from build123d import *

# Parameters (mm, degrees)
BASE_PLATE_DEPTH         = 12
LUG_DEPTH                = 35
BOSS_SKETCH_R            = 25
CYLINDRICAL_BOSS_DEPTH   = 45
LUG_FILLET_R6_R          = 6
MIRRORED_LUG_FILLET_R6_R = 6
BOSS_BORE_SKETCH_R       = 16
BOSS_BORE_DEPTH          = 131
SIDE_EAR_SKETCH_R        = 10.000000003
SIDE_EAR_DEPTH           = 10
RELIEF_CUT_SKETCH_R      = 5
RELIEF_CUT_DEPTH         = 10


with BuildPart() as part:
    # Base Plate Sketch → Base Plate (new body)
    with BuildSketch(Plane(origin=(0, 0, 0), x_dir=(1, 0, 0), z_dir=(0, 1, 0))):
        with BuildLine():
            Line((0, 0), (52.086042587, 0))
            Line((52.086042587, 0), (52.086042587, 34.268491931))
            ThreePointArc((52.086042587, 34.268491931), (55.457925039, 42.608491187), (63.678640518, 46.261574252))
            ThreePointArc((63.678640518, 46.261574252), (70.963844757, 49.044672415), (75, 55.717699243))
            Line((75, 55.717699243), (75, 83.735383518))
            Line((75, 83.735383518), (75, 93.85377774))
            Line((75, 93.85377774), (20.146433568, 93.85377774))
            Line((20.146433568, 93.85377774), (-75, 93.85377774))
            Line((-75, 93.85377774), (-75, 83.735383518))
            Line((-75, 83.735383518), (-75, 55.717699243))
            ThreePointArc((-75, 55.717699243), (-70.963844757, 49.044672415), (-63.678640518, 46.261574252))
            ThreePointArc((-63.678640518, 46.261574252), (-55.457925039, 42.608491187), (-52.086042587, 34.268491931))
            Line((-52.086042587, 34.268491931), (-52.086042587, 0))
            Line((-52.086042587, 0), (0, 0))
        make_face()
    extrude(amount=BASE_PLATE_DEPTH)

    # Lug Sketch → Lug (add)
    with BuildSketch(Plane(origin=(0, 12, 0), x_dir=(1, 0, 0), z_dir=(0, 1, 0))):
        with BuildLine():
            ThreePointArc((0.048175719, 53.923822509), (17.764829386, 46.622880149), (25.108500916, 28.923895292))
            Line((25.108500916, 28.923895292), (25.108500916, 53.923895292))
            ThreePointArc((25.108500916, 53.923895292), (25.987180573, 56.045215635), (28.108500916, 56.923895292))
            Line((28.108500916, 56.923895292), (31.814716412, 56.923895292))
            ThreePointArc((31.814716412, 56.923895292), (42.43838692, 63.34378553), (41.694924329, 75.734291134))
            Line((41.694924329, 75.734291134), (41.694924329, 83.85377774))
            Line((41.694924329, 83.85377774), (75, 83.85377774))
            Line((75, 83.85377774), (75, 93.85377774))
            Line((75, 93.85377774), (41.694924329, 93.85377774))
            Line((41.694924329, 93.85377774), (34.699589824, 93.85377774))
            Line((34.699589824, 93.85377774), (34.699589824, 83.85377774))
            Line((34.699589824, 83.85377774), (0.012065057, 83.85377774))
            Line((0.012065057, 83.85377774), (0.048175719, 53.923822509))
        make_face()
    lug = extrude(amount=LUG_DEPTH)

    # Lug Mirror: Lug across plane
    add(lug.mirror(Plane(origin=(0, 0, 0), x_dir=(0, 0, 1), z_dir=(1, 0, 0))))

    # Boss Sketch → Cylindrical Boss (add)
    with BuildSketch(Plane(origin=(0, 12, 0), x_dir=(1, 0, 0), z_dir=(0, 1, 0))):
        with Locations(Location((0.108500916, 28.923895292, 0), (0, 0, 90.138255303))):
            Circle(BOSS_SKETCH_R)
    extrude(amount=CYLINDRICAL_BOSS_DEPTH)

    # Lug Fillet R6
    lug_fillet_r6_edges = [part.edges().sort_by_distance(p)[0] for p in [
        (41.694924329, 29.5, -83.85377774),
    ]]
    fillet(lug_fillet_r6_edges, radius=LUG_FILLET_R6_R)

    # Mirrored Lug Fillet R6
    mirrored_lug_fillet_r6_edges = [part.edges().sort_by_distance(p)[0] for p in [
        (-41.694924329, 29.5, -83.85377774),
    ]]
    fillet(mirrored_lug_fillet_r6_edges, radius=MIRRORED_LUG_FILLET_R6_R)

    # Boss Bore Sketch → Boss Bore (cut)
    with BuildSketch(Plane(origin=(0, 57, 0), x_dir=(1, 0, 0), z_dir=(0, 1, 0))):
        with Locations(Location((0.108500916, 28.923895292, 0), (0, 0, 270))):
            Circle(BOSS_BORE_SKETCH_R)
    extrude(amount=-BOSS_BORE_DEPTH, mode=Mode.SUBTRACT)

    # Side Ear Sketch → Side Ear (add)
    with BuildSketch(Plane(origin=(52.086042587, 0, 0), x_dir=(0, 0, -1), z_dir=(1, 0, 0))):
        with BuildLine():
            Line((0, 0), (0, -9.993926671))
            Line((0, -9.993926671), (10.199483508, -69.224345425))
            ThreePointArc((10.199483505, -69.224345426), (28.923895292, -85.000000013), (47.648307078, -69.224345426))
            Line((47.648307075, -69.224345425), (56.277342763, -19.113827886))
            ThreePointArc((56.277342763, -19.113827886), (61.607291904, -7.474858686), (71.999618374, 0))
            Line((71.999618374, 0), (0, 0))
        make_face()
        with Locations((28.923895292, -66.00000001)):
            Circle(SIDE_EAR_SKETCH_R, mode=Mode.SUBTRACT)
    side_ear = extrude(amount=-SIDE_EAR_DEPTH)

    # Side Ear Mirror: Side Ear across plane
    add(side_ear.mirror(Plane(origin=(0, 0, 0), x_dir=(0, 0, 1), z_dir=(1, 0, 0))))

    # Relief Cut Sketch → Relief Cut (cut)
    with BuildSketch(Plane.XY.offset(-83.85377774)):
        with Locations((61.606022049, 35)):
            Circle(RELIEF_CUT_SKETCH_R)
        with Locations(Location((-61.606022049, 35, 0), (0, 0, 180))):
            Circle(RELIEF_CUT_SKETCH_R)
    extrude(amount=-RELIEF_CUT_DEPTH, mode=Mode.SUBTRACT)


solid = part.part
Work out the finished part from the listing and answer in its coordinate system (mm). A direction names the side the tool comes from. Give positions to 0.01 mm unless a question says otherwise; leave off trailing zeros. Write each loop counter-clockwise with the first axis right and the second up, starting at its lowest first coordinate (ties: lowest second). Pieces come first, ordered by that corner, then holes.
Q1. The part is cut by section D-D on z = -17. Give the vertices of the cut face in (x, y).
Answer:
outline: (-52.09, -80.79) - (-42.09, -80.79) - (-42.09, 0) - (-10.56, 0) - (-10.56, 57) - (-21.86, 57) - (-21.86, 12) - (-52.09, 12) - close; (10.78, 0) - (42.09, 0) - (42.09, -80.79) - (52.09, -80.79) - (52.09, 12) - (22.08, 12) - (22.08, 57) - (10.78, 57) - close
Q2. A tool of negligible diameter and unlimited length cuts with its end or side. For faces 1 (the face through (-25.109, 29, -41)), 2 (the face through (43.406, 29.745, -82.05)), 3 (the face through (-43.499, 29.745, -82.143)), from which of +Z, -Z, +X, -X, +Y, -Y can it reach the whole face along a straight path? Write none if from no direction.
Answer:
face 1: +Z, -X, +Y
face 2: +X, +Y
face 3: -X, +Y
Q3. Straight lines are drawn through the part: L1, parallel to X at y = 9, z = -28; L2, parallel to X at y = -18.5, z = -13; L3, parallel to Y at x = 31.5, z = -30. For each, find the intervals that lie inside material, in ascending order.
Answer:
L1: x = -52.09 to -15.86, 16.08 to 52.09
L2: x = -52.09 to -42.09, 42.09 to 52.09
L3: y = 0 to 12
Q4. Given pin 1 (18 mm diameter, centred on y = -66, z = -28.92, fed in from -X); pin 2 (6 mm diameter, centred on x = -51.5, y = 27.5, fed in from +Z); pin 3 (5 mm diameter, centred on x = 53.5, z = -36, fed in from +Y); pin 4 (3 mm diameter, centred on y = 11.5, z = -39.5, fed in from +X), each flat-ended and moving along its own axis, determine where each tip first touches the part or whether it passes through.
Answer:
pin 1: passes through
pin 2: stops at z = -83.85
pin 3: stops at y = 12
pin 4: stops at x = 54.15
Q5. The part is cut by section B-B on y = -66. Give the vertices of the cut face in (x, z).
Answer:
outline: (-52.09, -48.2) - (-42.09, -48.2) - (-42.09, -38.92) - (-52.09, -38.92) - close; (-52.09, -18.92) - (-42.09, -18.92) - (-42.09, -9.64) - (-52.09, -9.64) - close; (42.09, -48.2) - (52.09, -48.2) - (52.09, -38.92) - (42.09, -38.92) - close; (42.09, -18.92) - (52.09, -18.92) - (52.09, -9.64) - (42.09, -9.64) - close
Q6. The part is cut by section C-C on x = 13. Give the vertices of the cut face in (y, z).
Answer:
outline: (0, -93.85) - (12, -93.85) - (12, -83.85) - (47, -83.85) - (47, -50.34) - (57, -50.34) - (57, -38.4) - (0, -38.4) - close; (0, -19.45) - (57, -19.45) - (57, -7.5) - (12, -7.5) - (12, 0) - (0, 0) - close
Q7. For a pull along Y with two mould halves and no side action, classify faces 4 (the face through (-61, 29, -83.854)), 5 (the face through (-47.156, -59.242, -21.553)), 6 (the face through (29, 47, -76)) as released by +Y, released by -Y, zero draft, split by the parting line, or undercut.
Answer:
face 4: zero draft
face 5: undercut
face 6: released by +Y
Q8. The part is cut by section A-A on z = -37. State how many separate pieces and enclosed holes the cut face has, and give its area (3 significant figures).
Answer:
separate pieces: 4
enclosed holes: 0
area: 3,330 mm2
